The drawing under review shows one solid part. Ordinate dimensions are in mm from its lowest x, y, z. Give positions to 0.01 mm unless a question says otherwise; leave off trailing zeros. Write each loop counter-clockwise with the first axis right and the second up, starting at its lowest first coordinate (ties: lowest second). Pieces come first, ordered by that corner, then holes. Notation, with made-up numbers: (-9, 48.5) -> (47, 48.5) arc R26 cw to (47, 64.5) -> close; hole circle Ø10 at (70.5, -2.75). An arc over 180 degrees is marked (long way). Write item = value, one per line.
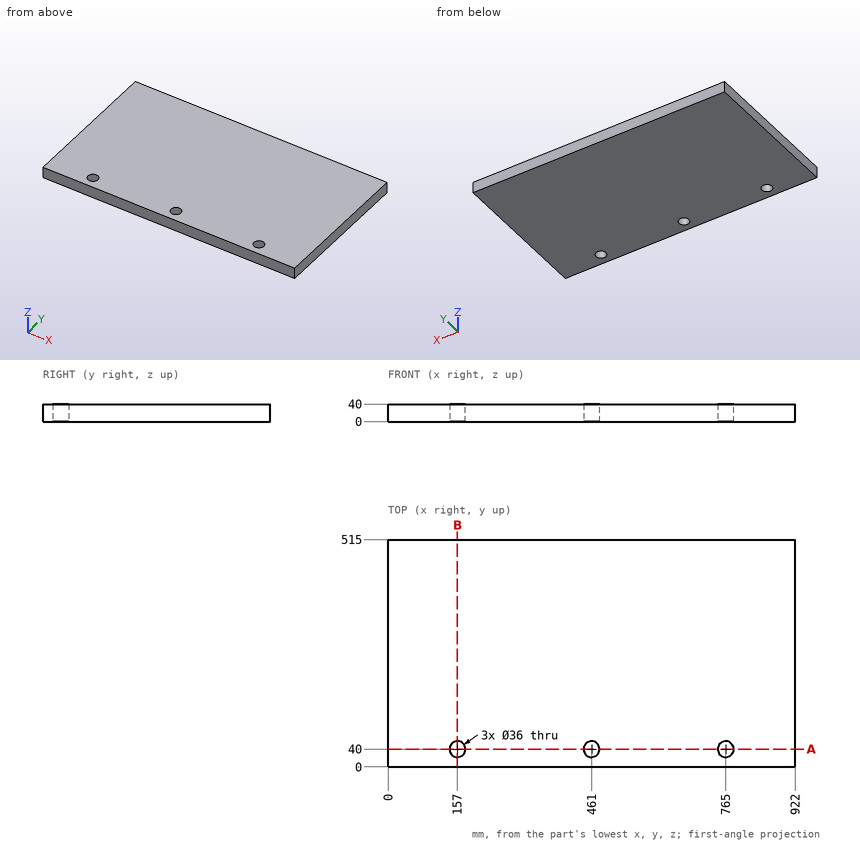
(1) Take a section at B-B (x = 157). Write out the cut boundary in (y, z).
Answers below:
outline = (0, 0) -> (22, 0) -> (22, 40) -> (0, 40) -> close; (58, 0) -> (515, 0) -> (515, 40) -> (58, 40) -> close
(2) Take a section at A-A (y = 40). Write out the cut boundary in (x, z).
Answers below:
outline = (0, 0) -> (139, 0) -> (139, 40) -> (0, 40) -> close; (175, 0) -> (443, 0) -> (443, 40) -> (175, 40) -> close; (479, 0) -> (747, 0) -> (747, 40) -> (479, 40) -> close; (783, 0) -> (922, 0) -> (922, 40) -> (783, 40) -> close
(3) For pin 1 (4 mm diameter, centred on y = 252.5, z = 15, fed in from -X); pin 2 (21.5 mm diameter, centred on x = 157, y = 40, fed in from +Z) (1 decimal), all flat-tipped, find the tip position at first contact; note any pin that passes through.
Answers below:
pin_1 = 0
pin_2 = through
(4) To check wall thickness, follow probe 1 along Y at (x, z) = (461, 22); probe 2 along X at (y, z) = (28, 24); probe 3 along X at (y, z) = (54.5, 18). State the ranges of each line that lie inside material, in increasing order.
Answers below:
probe_1 = 0 to 22, 58 to 515
probe_2 = 0 to 143.58, 170.42 to 447.58, 474.42 to 751.58, 778.42 to 922
probe_3 = 0 to 146.33, 167.67 to 450.33, 471.67 to 754.33, 775.67 to 922
